from build123d import *

# Parameters (mm, degrees)
SKETCH3_W          = 20
SKETCH3_H          = 43.741822135
CUT_EXTRUDE1_DEPTH = 374.22982196
LPATTERN1_COUNT    = 7
LPATTERN1_PITCH    = 37.5


with BuildPart() as part:
    # Sketch1 → Revolve1 (revolve)
    with BuildSketch(Plane.XY, mode=Mode.PRIVATE) as revolve1_sk:
        Polygon((0, 37.5), (-140, 37.5), (-140, 120), (-140, 174.5), (140, 174.5), (140, 120), (0, 120), align=None)
    revolve(revolve1_sk.sketch.rotate(Axis((0, 0, 0), (1, 0, 0)), 90), axis=Axis((0, 0, 0), (1, 0, 0)))

    # Sketch2 → Cut-Revolve1 (revolve, cut)
    with BuildSketch(Plane(origin=(0, 0, 0), x_dir=(1, 0, 0), z_dir=(0, 1, 0)), mode=Mode.PRIVATE) as cut_revolve1_sk:
        Polygon((-131.080105661, 181.63495756), (-119.501606075, 146), (-105.498393925, 146), (-93.919894339, 181.63495756), align=None)
    cut_revolve1 = revolve(cut_revolve1_sk.sketch.rotate(Axis((-238.897121458, 0, 0), (1, 0, 0)), 180), axis=Axis((-238.897121458, 0, 0), (1, 0, 0)), mode=Mode.SUBTRACT)

    # Sketch3 → Cut-Extrude1 (cut, through all)
    with BuildSketch(Plane.ZY.offset(140)):
        with Locations((0, 20.529088933)):
            Rectangle(SKETCH3_W, SKETCH3_H)
    extrude(amount=-CUT_EXTRUDE1_DEPTH, mode=Mode.SUBTRACT)

    # LPattern1: Cut-Revolve1 ×7
    with Locations(*[(i * LPATTERN1_PITCH, 0, 0) for i in range(1, LPATTERN1_COUNT)]):
        add(cut_revolve1, mode=Mode.SUBTRACT)


solid = part.part
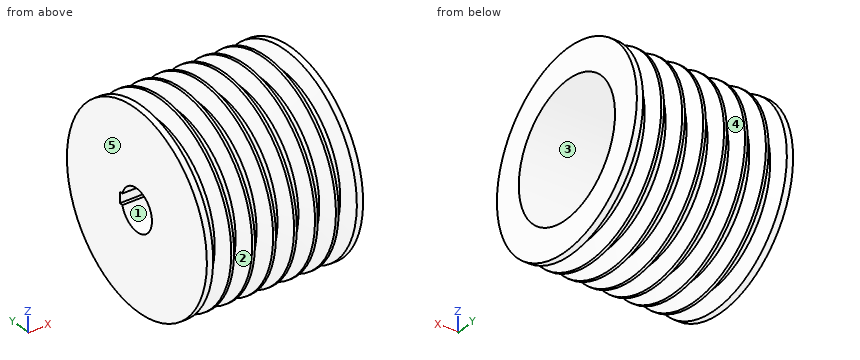
Verification items for the finished model (mm, model axes). Face numbers are marked on the shaded views. A direction names the side the tool comes from. Coordinates: 2 decimals unless noted, no trailing zeros. Order: outer loops, then holes, each group sorted by start corner. A loop starts at its lowest first (then second) coordinate and runs counter-clockwise, first axis right, second up.
1. Sectioned sample at A-A, the plane x = -113. Record the cut outline in (y, z), and give its area (3 significant figures).
Results found:
outline: circle Ø292 at (0, 0); hole (36.14, -10) - (42.4, -10) - (42.4, 10) - (36.14, 10) arc R37.5 ccw (long way) to start
area: 62,400 mm2
2. Scan lines: line 1 (Y direction, x = 43, z = 0); line 2 (X direction, y = -69.5, z = -79.5); line 3 (Y direction, x = 106, z = 103.5). Record each from-to range of solid material in increasing order.
Results found:
line 1: y = -146 to -120, 120 to 146
line 2: x = -140 to 0
line 3: y = -102.97 to -60.73, 60.73 to 102.97
3. Release check for a two-part mould opening along Y. For the marked faces 3, 4 and 5 record: +Y half, -Y half, draft (parallel to the pull), parting line (faces both ways), or undercut.
Results found:
face 3: undercut
face 4: parting line
face 5: draft
4. Go/stop test with flat-tipped pins: pin 1 Ø5 at (x, y) = (21, 70) entering from -Z; pin 2 Ø6 at (x, z) = (59.5, 6.5) entering from -Y; pin 3 Ø8 at (y, z) = (-10.5, 45.5) entering from +X. Record where each tip stops, or that it passes through.
Results found:
pin 1: stops at z = -160.92
pin 2: stops at y = -174.46
pin 3: stops at x = 0
5. Set-up check for the marked faces 1 and 2: record each of +Z, -Z, +X, -X, +Y, -Y from which the full face is reachable in a straight line by a thin tool's end or side.
Results found:
face 1: +X, -X
face 2: none
